Geometry: final body of the model. Coordinates: model frame, mm. Face numbers are marked on the shaded views. A direction names the side the tool comes from. Give positions to 0.01 mm unless a question says otherwise; leave off trailing zeros. Order: outer loops, then holes, each group sorted by start corner. A loop starts at its lowest first (then second) coordinate and runs counter-clockwise, first axis right, second up. Notation, with made-up numbers: (0, -11) -> (24, -11) arc R21 ccw to (24, -4) -> close; hole circle Ø11 at (41.25, -6.5). An arc over 180 degrees is marked (long way). One line per question, with ' | ' between items.
from build123d import *

# Parameters (mm, degrees)
STEPPED_BLOCK_BODY_DEPTH         = 65
RELIEF_CUT_20X20_DEPTH           = 200.562020435
ARC_CUT_115_SKETCH_R             = 115
ARC_CUT_115_DEPTH                = 12
ARC_CUT_170_SKETCH_R             = 170
ARC_CUT_170_DEPTH                = 40
LOWER_C_BORE_HOLE_20_D           = 20
LOWER_C_BORE_HOLE_20_DEPTH       = 99.874921777
LOWER_C_BORE_HOLE_20_CBORE_D     = 30
LOWER_C_BORE_HOLE_20_CBORE_DEPTH = 9
HOLE_CLEARANCE_NOTCH_SKETCH_R    = 15
HOLE_CLEARANCE_NOTCH_DEPTH       = 12


with BuildPart() as part:
    # Stepped Profile Sketch → Stepped Block Body (new body)
    with BuildSketch(Plane.XY):
        Polygon((0, 0), (0, 75), (14.43375673, 100), (65, 100), (65, 60), (53, 60), (53, 48), (65, 48), (125, 48), (125, 36), (160, 36), (160, 0), (100, 0), (100, -5), (70, -5), (70, 0), align=None)
    extrude(amount=STEPPED_BLOCK_BODY_DEPTH)

    # Relief Cut Sketch → Relief Cut 20x20 (cut, through all)
    with BuildSketch(Plane(origin=(160, 0, 0), x_dir=(0, 0, -1), z_dir=(1, 0, 0))):
        Polygon((-45, 0), (-45, 5), (-20, 5), (-20, 0), (-20, -9.038328121), (-45, -9.038328121), align=None)
    extrude(amount=-RELIEF_CUT_20X20_DEPTH, mode=Mode.SUBTRACT)

    # Arc Cut 115 Sketch → Arc Cut 115 (cut)
    with BuildSketch(Plane(origin=(0, 48, 0), x_dir=(1, 0, 0), z_dir=(0, 1, 0))):
        with Locations((235.312057365, -32.5)):
            Circle(ARC_CUT_115_SKETCH_R)
    extrude(amount=-ARC_CUT_115_DEPTH, mode=Mode.SUBTRACT)

    # Arc Cut 170 Sketch → Arc Cut 170 (cut)
    with BuildSketch(Plane(origin=(0, 100, 0), x_dir=(1, 0, 0), z_dir=(0, 1, 0))):
        with Locations((231.86446596, -32.5)):
            Circle(ARC_CUT_170_SKETCH_R)
    extrude(amount=-ARC_CUT_170_DEPTH, mode=Mode.SUBTRACT)

    # Sketch11 → Upper C-Bore Hole Ø20 (revolve, cut)
    with BuildSketch(Plane(origin=(125, 36, 32.5), x_dir=(0, 0, 1), z_dir=(1, 0, 0))):
        Polygon((0, 0), (0, 99.874921777), (10, 99.874921777), (10, 9), (15, 9), (15, 0), align=None)
    revolve(axis=Axis((125, -74, 32.5), (0, 1, 0)), mode=Mode.SUBTRACT)

    # Lower C-Bore Hole Ø20
    with Locations(Plane(origin=(35, 100, 32.5), x_dir=(1, 0, 0), z_dir=(0, 1, 0))):
        with Locations((0, 0)):
            CounterBoreHole(LOWER_C_BORE_HOLE_20_D / 2, LOWER_C_BORE_HOLE_20_CBORE_D / 2, LOWER_C_BORE_HOLE_20_CBORE_DEPTH, depth=LOWER_C_BORE_HOLE_20_DEPTH)

    # Hole Clearance Notch Sketch → Hole Clearance Notch (cut)
    with BuildSketch(Plane(origin=(0, 48, 0), x_dir=(1, 0, 0), z_dir=(0, 1, 0))):
        with Locations(Location((125, -32.5, 0), (0, 0, 270))):
            Circle(HOLE_CLEARANCE_NOTCH_SKETCH_R)
    extrude(amount=-HOLE_CLEARANCE_NOTCH_DEPTH, mode=Mode.SUBTRACT)


solid = part.part
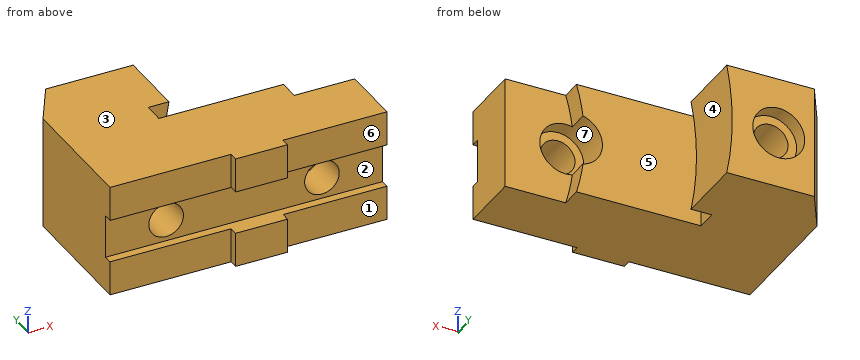
1) Set-up query: the marked faces 4, 5, 6 and 7. Return all of +Z, -Z, +X, -X, +Y, -Y with unobstructed straight access to the full face (end or side cutting, diameter ignored); none if empty.
Check result:
face 4: +X, +Y | face 5: +Z, -Z, +X | face 6: +Z, -Z, +X, -Y | face 7: +Y
2) Section C-C on y = 43.5. Return loops of the section in (x, z).
Check result:
outline: (0, 0) -> (125, 0) arc R115 cw to (121.23, 17.98) arc R15 cw to (121.23, 47.02) arc R115 cw to (125, 65) -> (0, 65) -> close; hole circle Ø20 at (35, 32.5)
3) Pull-direction query (Z, two-part tool) for the marked faces 1, 2 and 3; classes: +Z half, -Z half, draft (parallel to the pull), parting line (faces both ways), or undercut.
Check result:
face 1: draft | face 2: undercut | face 3: +Z half
4) Section D-D on y = 18. Return loops of the section in (x, z), plus the area to 3 significant figures.
Check result:
outline: (0, 0) -> (160, 0) -> (160, 65) -> (0, 65) -> close; hole circle Ø20 at (35, 32.5); hole circle Ø20 at (125, 32.5) | area: 9,770 mm^2
5) Section B-B on z = 32.5. Return loops of the section in (x, y), plus the area to 3 significant figures.
Check result:
outline: (0, 5) -> (25, 5) -> (25, 91) -> (20, 91) -> (20, 100) -> (14.43, 100) -> (0, 75) -> close; (45, 5) -> (115, 5) -> (115, 27) -> (110, 27) -> (110, 48) -> (53, 48) -> (53, 60) -> (61.86, 60) -> (61.86, 100) -> (50, 100) -> (50, 91) -> (45, 91) -> close; (135, 5) -> (160, 5) -> (160, 36) -> (140, 36) -> (140, 27) -> (135, 27) -> close | area: 6,510 mm^2
6) Material intervals for probe 1 along X at (y, z) = (16, 32); probe 2 along Z at (x, y) = (35, 94); probe 3 along Y at (x, z) = (57, 12), sorted ascending. Write a range as from..to.
Check result:
probe 1: x = 0..25.01, 44.99..115.01, 134.99..160 | probe 2: z = 0..17.5, 47.5..65 | probe 3: y = 0..48, 60..100
7) Section A-A on x = 35. Return loops of the section in (y, z), plus the area to 4 significant figures.
Check result:
outline: (0, 0) -> (100, 0) -> (100, 17.5) -> (91, 17.5) -> (91, 22.5) -> (5, 22.5) -> (5, 20) -> (0, 20) -> close; (0, 45) -> (5, 45) -> (5, 42.5) -> (91, 42.5) -> (91, 47.5) -> (100, 47.5) -> (100, 65) -> (0, 65) -> close | area: 4,385 mm^2
8) Contact query for flat-ended pins moving along their axis: pin 1 Ø18 at (x, z) = (35, 32.5) entering from +Y; pin 2 Ø1.5 at (y, z) = (34.5, 11) entering from -X; pin 3 Ø6 at (y, z) = (55, 35.5) entering from +X; pin 4 Ø2.5 at (y, z) = (-2.5, 8) entering from -X. Output: stop coordinate, or through.
Check result:
pin 1: passes through | pin 2: stops at x = 0 | pin 3: stops at x = 53 | pin 4: stops at x = 70
